Geometry: final body of the model. Coordinates: model frame, mm. Face numbers are marked on the shaded views. A direction names the side the tool comes from. Round coordinates to 2 decimals unless told otherwise and drop trailing zeros. Loops run counter-clockwise (first coordinate to the right, second up) from the corner with the lowest first, then second, coordinate; pieces in that order, holes last. Notation, with made-up numbers: (36, 54) - (90, 54) arc R30 ccw to (90, 90) - close; hole circle Ø2 at (-32, 41). An arc over 180 degrees is marked (long way). Use CSV: the item, a comma, the result in double quotes.
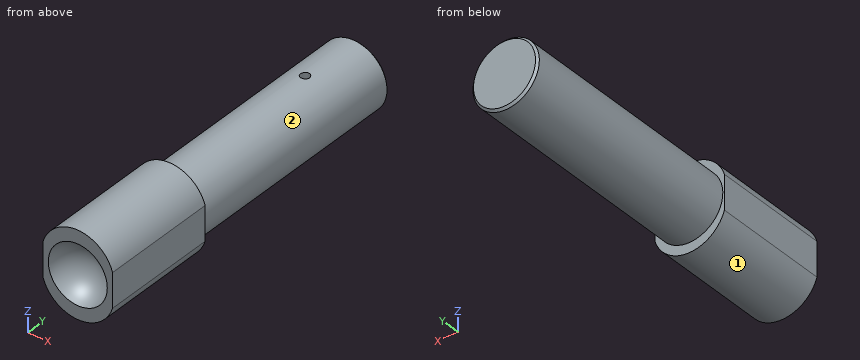
from build123d import *

# Parameters (mm, degrees)
EXTRUDE_1_DEPTH         = 110
SKETCH_2_R              = 31
EXTRUDE_2_DEPTH         = 220
HOLE_WIZARD_M10_1_D     = 8.5
HOLE_WIZARD_M10_1_DEPTH = 27.5
HOLE_WIZARD_M10_1_TIP   = 2.553657631
CHAMFER_1_SIZE          = 2


with BuildPart() as part:
    # 草图1 → 凸台-拉伸1 (new body)
    with BuildSketch(Plane(origin=(0, 0, 0), x_dir=(1, 0, 0), z_dir=(0, 1, 0))):
        with BuildLine():
            Line((32.5, -15.987492178), (32.5, 15.987492178))
            ThreePointArc((32.5, 15.987492178), (0, 40), (-32.5, 15.987492178))
            Line((-32.5, 15.987492178), (-32.5, -15.987492178))
            ThreePointArc((-32.5, -15.987492178), (0, -40), (32.5, -15.987492178))
        make_face()
    extrude(amount=EXTRUDE_1_DEPTH)

    # 草图2 → 凸台-拉伸2 (add)
    with BuildSketch(Plane(origin=(0, 110, 0), x_dir=(1, 0, 0), z_dir=(0, 1, 0))):
        with Locations(Location((0, 0, 0), (0, 0, 270))):
            Circle(SKETCH_2_R)
    extrude(amount=EXTRUDE_2_DEPTH)

    # M10 螺纹孔1
    with Locations(Plane.XY.offset(31)):
        with Locations((0, 270)):
            Hole(HOLE_WIZARD_M10_1_D / 2, depth=HOLE_WIZARD_M10_1_DEPTH)
            with Locations((0, 0, -(HOLE_WIZARD_M10_1_DEPTH + HOLE_WIZARD_M10_1_TIP / 2))):  # 118° drill point
                Cone(0, HOLE_WIZARD_M10_1_D / 2, HOLE_WIZARD_M10_1_TIP, mode=Mode.SUBTRACT)

    # 倒角1
    chamfer_1_edges = [part.edges().sort_by_distance(p)[0] for p in [
        (0, 330, -31),
    ]]
    chamfer(chamfer_1_edges, length=CHAMFER_1_SIZE)

    # 草图5 → 切除-旋转1 (revolve, cut)
    with BuildSketch(Plane.XY):
        with BuildLine():
            Line((0, 23), (0, -33))
            ThreePointArc((0, -33), (28, -5), (0, 23))
        make_face()
    revolve(axis=Axis((0, 23, 0), (0, -1, 0)), mode=Mode.SUBTRACT)


solid = part.part
Item 1: Pin query (flat end, axial travel): P1, Ø3, axis at y = 175, z = -20, coming from the -X side; P2, Ø2, axis at x = -3.5, y = 116, coming from the -Z side; P3, Ø7.5, axis at x = 0, y = 270, coming from the +Z side. Return the tip coordinate at first contact, or that it passes through.
Final values:
P1,"stops at x = -24.87"
P2,"stops at z = -30.9"
P3,"stops at z = 3.2"
Item 2: Section B-B on y = 154. Return the cut outline in (x, z), plus the area to 3 significant figures.
Final values:
outline,"circle Ø62 at (0, 0)"
area,"3,020 mm²"
Item 3: Reachability of the marked faces 1 and 2 from +Z, -Z, +X, -X, +Y, -Y: full face, straight path, thin tool, end or side. Return the list, or none.
Final values:
face 1,"-Z, +Y, -Y"
face 2,"+Y"
Item 4: Material intervals for line 1 (X direction, y = 270, z = 18); line 2 (X direction, y = 270, z = 16.5); line 3 (Y direction, x = 0, z = 15), sorted ascending.
Final values:
line 1,"x = -25.24 to -4.25, 4.25 to 25.24"
line 2,"x = -26.24 to -4.25, 4.25 to 26.24"
line 3,"y = 18.64 to 265.75, 274.25 to 330"
Item 5: Section A-A on y = 45.5. Return the cut outline in (x, z).
Final values:
outline,"(-32.5, -15.99) arc R34 ccw to (32.5, -15.99) - (32.5, 15.99) arc R34 ccw to (-32.5, 15.99) - close"
